Model file for the job. Use its own axes, mm. A direction names the side the tool comes from. Round coordinates to 2 decimals unless told otherwise and drop trailing zeros. Order: outer loops, then holes, each group sorted by start corner. A loop starts at its lowest first (then second) coordinate and runs counter-clockwise, first axis right, second up. Notation, with made-up numbers: (-27.75, 2) -> (-14.75, 2) arc R18 cw to (-14.75, 6) -> close; hole circle Ø2 at (49, 4.5). An arc over 180 degrees is marked (long way). Put each result on its own line as item: value. Start each with the question number.
Q1. Cut at A-A, the plane y = 45. List the corners of the cut face in (x, z) (3 decimals), and give its area (3 significant figures).
Q2. Probe L1, parallel to Y at x = -50.5, z = -6; L2, parallel to X at y = 59, z = -25.5; L3, parallel to Y at x = 24, z = -7.5. List the from-to ranges inside material, lowest first.
Q3. Cut at B-B, the plane y = 69.5. List the corners of the cut face in (x, z).
Q4. Cut at C-C, the plane x = 11. State how many separate pieces and enclosed holes the cut face has, and give its area (3 significant figures).
Q5. Pull direction Z, two halves, no side cores. Call faces 6 (the face through (-1, 10, -1)), 7 (the face through (-9.38, 31.247, -34.584)), 8 (the face through (0, 75, -1)): released by +Z, released by -Z, zero draft, split by the parting line, or undercut.
Q6. Flat gauge pins, fed straight in: P1, Ø4, axis at x = 3, y = 12.5, coming from the -Z side; P2, Ø10, axis at x = -40.5, z = -46, coming from the +Y side; P3, Ø12, axis at x = -38.5, y = 18, coming from the +Z side. Where does each tip first touch, or does it go through?
Q7. 3-axis set-ups, long thin cutter, end or side, ignore diameter. For faces 1 (the face through (-34.641, 31, -9)), 2 (the face through (-7.037, -0.22, 52.184)), 3 (the face through (-1, -15, -1)), 4 (the face through (-49, 0, -20)), 5 (the face through (34.641, 31, 9)): which of +Z, -Z, +X, -X, +Y, -Y reach the whole face in a straight line?
from build123d import *

# Parameters (mm, degrees)
HEX_BASE_DEPTH          = 15
SIDE_SLOT_1_20X10_DEPTH = 161.7015868
SIDE_SLOT_2_20X10_DEPTH = 176
SIDE_SLOT_3_20X10_DEPTH = 176
HEX_BOSS_DEPTH          = 60
CROSS_HOLE_1_SKETCH_R   = 15.75
CROSS_HOLE_1_31_5_DEPTH = 152.079449297
CROSS_HOLE_2_SKETCH_R   = 15.75
CROSS_HOLE_2_31_5_DEPTH = 159.823801743
CROSS_HOLE_3_SKETCH_R   = 15.75
CROSS_HOLE_3_31_5_DEPTH = 159.823801743


with BuildPart() as part:
    # Hex Base Sketch → Hex Base (new, symmetric)
    with BuildSketch(Plane(origin=(0, 0, 0), x_dir=(1, 0, 0), z_dir=(0, 1, 0))):
        Polygon((69.282032303, -40), (69.282032303, 40), (0, 80), (-69.282032303, 40), (-69.282032303, -40), (0, -80), align=None)
    extrude(amount=HEX_BASE_DEPTH, both=True)

    # Side Slot 1 Sketch → Side Slot 1 20x10 (cut, through all)
    with BuildSketch(Plane.ZY.offset(69.282032303)):
        with BuildLine():
            Line((-10, 10), (10, 10))
            ThreePointArc((10, 10), (20, 0), (10, -10))
            Line((10, -10), (-10, -10))
            ThreePointArc((-10, -10), (-20, 0), (-10, 10))
        make_face()
    extrude(amount=-SIDE_SLOT_1_20X10_DEPTH, mode=Mode.SUBTRACT)

    # Side Slot 2 Sketch → Side Slot 2 20x10 (cut, through all)
    with BuildSketch(Plane(origin=(34.641016151, 0, -60), x_dir=(-0.8660254037844386, 0, -0.5000000000000003), z_dir=(0.5000000000000002, 0, -0.8660254037844385))):
        with BuildLine():
            Line((-10, 10), (10, 10))
            ThreePointArc((10, 10), (20, 0), (10, -10))
            Line((10, -10), (-10, -10))
            ThreePointArc((-10, -10), (-20, 0), (-10, 10))
        make_face()
    extrude(amount=-SIDE_SLOT_2_20X10_DEPTH, mode=Mode.SUBTRACT)

    # Side Slot 3 Sketch → Side Slot 3 20x10 (cut, through all)
    with BuildSketch(Plane(origin=(-34.641016151, 0, -60), x_dir=(-0.8660254037844388, 0, 0.49999999999999983), z_dir=(-0.4999999999999998, 0, -0.8660254037844387))):
        with BuildLine():
            Line((-10, 10), (10, 10))
            ThreePointArc((10, 10), (20, 0), (10, -10))
            Line((10, -10), (-10, -10))
            ThreePointArc((-10, -10), (-20, 0), (-10, 10))
        make_face()
    extrude(amount=-SIDE_SLOT_3_20X10_DEPTH, mode=Mode.SUBTRACT)

    # Hex Boss Sketch → Hex Boss (add)
    with BuildSketch(Plane(origin=(0, 15, 0), x_dir=(1, 0, 0), z_dir=(0, 1, 0))):
        Polygon((34.641016151, -20), (34.641016151, 20), (0, 40), (-34.641016151, 20), (-34.641016151, -20), (0, -40), align=None)
    extrude(amount=HEX_BOSS_DEPTH)

    # Cross Hole 1 Sketch → Cross Hole 1 Ø31.5 (cut, through all)
    with BuildSketch(Plane(origin=(34.641016151, 0, 0), x_dir=(0, 0, -1), z_dir=(1, 0, 0))):
        with Locations((0, 45)):
            Circle(CROSS_HOLE_1_SKETCH_R)
    extrude(amount=-CROSS_HOLE_1_31_5_DEPTH, mode=Mode.SUBTRACT)

    # Cross Hole 2 Sketch → Cross Hole 2 Ø31.5 (cut, through all)
    with BuildSketch(Plane(origin=(17.320508076, 0, -30), x_dir=(-0.8660254037844384, 0, -0.5000000000000004), z_dir=(0.5000000000000004, 0, -0.8660254037844384))):
        with Locations((0, 45)):
            Circle(CROSS_HOLE_2_SKETCH_R)
    extrude(amount=-CROSS_HOLE_2_31_5_DEPTH, mode=Mode.SUBTRACT)

    # Cross Hole 3 Sketch → Cross Hole 3 Ø31.5 (cut, through all)
    with BuildSketch(Plane(origin=(17.320508076, 0, 30), x_dir=(0.8660254037844388, 0, -0.4999999999999997), z_dir=(0.4999999999999997, 0, 0.8660254037844388))):
        with Locations((0, 45)):
            Circle(CROSS_HOLE_3_SKETCH_R)
    extrude(amount=-CROSS_HOLE_3_31_5_DEPTH, mode=Mode.SUBTRACT)


solid = part.part
Ans:
1. outline: (-34.641, -20) -> (-30.96, -22.125) -> (-27.28, -15.75) -> (-34.641, -15.75) -> close; (-34.641, 15.75) -> (-27.28, 15.75) -> (-30.96, 22.125) -> (-34.641, 20) -> close; (-3.681, -37.875) -> (0, -40) -> (3.681, -37.875) -> (0, -31.5) -> close; (-3.681, 37.875) -> (0, 31.5) -> (3.681, 37.875) -> (0, 40) -> close; (27.28, -15.75) -> (30.96, -22.125) -> (34.641, -20) -> (34.641, -15.75) -> close; (27.28, 15.75) -> (34.641, 15.75) -> (34.641, 20) -> (30.96, 22.125) -> close
1. area: 188 mm^2
2. L1: y = -15 to -10, 10 to 15
2. L2: x = -25.11 to -23.05, -6.39 to 6.39, 23.05 to 25.11
2. L3: y = -15 to -10, 10 to 31.15, 58.85 to 75
3. outline: (-34.64, -20) -> (0, -40) -> (34.64, -20) -> (34.64, 20) -> (0, 40) -> (-34.64, 20) -> close
4. separate pieces: 2
4. enclosed holes: 1
4. area: 4,210 mm^2
5. face 6: undercut
5. face 7: released by -Z
5. face 8: zero draft
6. P1: stops at z = -79.42
6. P2: stops at y = 15
6. P3: stops at z = 60.77
7. face 1: +Z, -Z, -X, +Y
7. face 2: none
7. face 3: +Z, -Z, +X, -X, -Y
7. face 4: +X, -X
7. face 5: +Z, -Z, +X, +Y
